```python
from build123d import *

# Parameters (mm, degrees)
FLANGE_PLATE_PROFILE_R       = 6.25
FLANGE_PLATE_PROFILE_R_2     = 12.5
FLANGE_PLATE_20MM_DEPTH      = 20
HUB_PROFILE_90_70_R          = 45
HUB_PROFILE_90_70_R_2        = 35
HUB_90X60_DEPTH              = 60
INNER_BOSS_PROFILE_70_30_R   = 35
INNER_BOSS_PROFILE_70_30_R_2 = 15
INNER_BOSS_70_BORE_30_DEPTH  = 40


with BuildPart() as part:
    # Flange Plate Profile → Flange Plate 20mm (new body)
    with BuildSketch(Plane.XY):
        with BuildLine():
            Line((-4, 9.16515139), (80, 45.82575695))
            ThreePointArc((80, 45.82575695), (97.330664824, 49.928695654), (115, 47.696960071))
            Line((115, 47.696960071), (206, 19.078784028))
            ThreePointArc((206, 19.078784028), (220, 0), (206, -19.078784028))
            Line((206, -19.078784028), (115, -47.696960071))
            ThreePointArc((115, -47.696960071), (97.330664824, -49.928695654), (80, -45.82575695))
            Line((80, -45.82575695), (-4, -9.16515139))
            ThreePointArc((-4, -9.16515139), (-10, 0), (-4, 9.16515139))
        make_face()
        Circle(FLANGE_PLATE_PROFILE_R, mode=Mode.SUBTRACT)
        with Locations((200, 0)):
            Circle(FLANGE_PLATE_PROFILE_R_2, mode=Mode.SUBTRACT)
    extrude(amount=FLANGE_PLATE_20MM_DEPTH)

    # Hub Profile Ø90-Ø70 → Hub Ø90x60 (add)
    with BuildSketch(Plane.XY.offset(20)):
        with Locations((100, 0)):
            Circle(HUB_PROFILE_90_70_R)
        with Locations((100, 0)):
            Circle(HUB_PROFILE_90_70_R_2, mode=Mode.SUBTRACT)
    extrude(amount=HUB_90X60_DEPTH)

    # Inner Boss Profile Ø70-Ø30 → Inner Boss Ø70 Bore Ø30 (add)
    with BuildSketch(Plane.XY.offset(20)):
        with Locations((100, 0)):
            Circle(INNER_BOSS_PROFILE_70_30_R)
        with Locations((100, 0)):
            Circle(INNER_BOSS_PROFILE_70_30_R_2, mode=Mode.SUBTRACT)
    extrude(amount=INNER_BOSS_70_BORE_30_DEPTH)


solid = part.part
```
Source: CAD feature listing. Evaluate the final solid. Frame: model axes, mm. A direction names the side the tool comes from. Coordinates: 2 decimals unless noted, no trailing zeros. Write each loop counter-clockwise with the first axis right and the second up, starting at its lowest first coordinate (ties: lowest second). Pieces come first, ordered by that corner, then holes. Notation, with made-up numbers: (47, 67) -> (90, 67) arc R20 cw to (90, 73) -> close; hole circle Ø7 at (78, -6.5). An arc over 180 degrees is marked (long way). Return JSON: item names as keys, results as strings. Group by question number.
1) Section query C-C, the plane z = 10. Return loops of the section in (x, y).
2) Section query B-B, the plane x = 195. Return loops of the section in (y, z).
3) Mould query, pull axis X, two halves, no side actions, for faces 1 (the face through (159.86, 33.59, 9.86)), 2 (the face through (100, 0, 20)), 3 (the face through (37.41, 27.24, 9.86)). Classes: +X half, -X half, draft (parallel to the pull), parting line (faces both ways), or undercut.
4) Contact query for flat-ended pins moving along their axis: P1, Ø5, axis at x = 102, z = 36.5, coming from the +Y side; P2, Ø10, axis at x = 0, y = 0, coming from the +Z side; P3, Ø2, axis at x = 178, y = 13, coming from the +Z side; P4, Ø24, axis at x = 94.5, y = 7, coming from the +Z side. Output: stop coordinate, or through.
5) Section query A-A, the plane y = 0. Return loops of the section in (x, z).
6) Set-up query: faces 4 (the face through (161.1, -33.2, 9.9)), 5 (the face through (132, 34, 20)). Return all of +Z, -Z, +X, -X, +Y, -Y with unobstructed straight access to the full face (end or side cutting, diameter ignored); none if empty.
7) Ray query, line 1 along Y through (x, z) = (100, 48.5); line 2 along Y through (x, z) = (100, 73.75); line 3 along Z through (x, y) = (126, -21.5). Return the intervals inside material, ascending.
8) Section query D-D, the plane z = 68. Return loops of the section in (x, y), plus the area to 3 significant figures.
From the geometry:
{
 "1": {"outline": "(-4, -9.17) -> (80, -45.83) arc R50 ccw to (115, -47.7) -> (206, -19.08) arc R20 ccw to (206, 19.08) -> (115, 47.7) arc R50 ccw to (80, 45.83) -> (-4, 9.17) arc R10 ccw to start; hole circle Ø12.5 at (0, 0); hole circle Ø25 at (200, 0)"},
 "2": {"outline": "(-22.54, 0) -> (-11.46, 0) -> (-11.46, 20) -> (-22.54, 20) -> close; (11.46, 0) -> (22.54, 0) -> (22.54, 20) -> (11.46, 20) -> close"},
 "3": {"face 1": "+X half", "face 2": "undercut", "face 3": "-X half"},
 "4": {"P1": "y = 45", "P2": "through", "P3": "z = 20", "P4": "z = 60"},
 "5": {"outline": "(-10, 0) -> (-6.25, 0) -> (-6.25, 20) -> (-10, 20) -> close; (6.25, 0) -> (187.5, 0) -> (187.5, 20) -> (145, 20) -> (145, 80) -> (135, 80) -> (135, 60) -> (115, 60) -> (115, 20) -> (85, 20) -> (85, 60) -> (65, 60) -> (65, 80) -> (55, 80) -> (55, 20) -> (6.25, 20) -> close; (212.5, 0) -> (220, 0) -> (220, 20) -> (212.5, 20) -> close"},
 "6": {"face 4": "+Z, -Z, +X, -Y", "face 5": "+Z"},
 "7": {"line 1": "-45 to -15, 15 to 45", "line 2": "-45 to -35, 35 to 45", "line 3": "0 to 60"},
 "8": {"outline": "circle Ø90 at (100, 0); hole circle Ø70 at (100, 0)", "area": "2,510 mm²"}
}
